from build123d import *

# Parameters (mm, degrees)
SKETCH2_R               = 32.5
CUT_EXTRUDE1_DEPTH      = 50
SKETCH3_R               = 30
CUT_EXTRUDE2_DEPTH      = 287.147252302
CHAMFER1_SIZE           = 1.5
CHAMFER2_SIZE           = 1.5
CUT_EXTRUDE3_DEPTH      = 336.306203343
CUT_EXTRUDE3_DEPTH_BACK = 336.306203343
SKETCH4_R               = 4
SKETCH7_W               = 2.1
SKETCH7_H               = 40


with BuildPart() as part:
    # Sketch1 → Revolve1 (revolve)
    with BuildSketch(Plane.XY, mode=Mode.PRIVATE) as revolve1_sk:
        Polygon((0, 0), (0, 37.5), (25, 37.5), (25, 36.5), (28, 36.5), (28, 38), (30, 38), (30, 40), (330.5, 40), (330.5, 0), align=None)
    revolve(revolve1_sk.sketch.rotate(Axis((0, 0, 0), (-1, 0, 0)), 90), axis=Axis((0, 0, 0), (-1, 0, 0)))

    # Sketch2 → Cut-Extrude1 (cut)
    with BuildSketch(Plane(origin=(330.5, 0, 0), x_dir=(0, 0, -1), z_dir=(1, 0, 0))):
        Circle(SKETCH2_R)
    extrude(amount=-CUT_EXTRUDE1_DEPTH, mode=Mode.SUBTRACT)

    # Sketch3 → Cut-Extrude2 (cut, through all)
    with BuildSketch(Plane(origin=(280.5, 0, 0), x_dir=(0, 0, -1), z_dir=(1, 0, 0))):
        Circle(SKETCH3_R)
    extrude(amount=-CUT_EXTRUDE2_DEPTH, mode=Mode.SUBTRACT)

    # Chamfer1
    chamfer1_edges = [part.edges().sort_by_distance(p)[0] for p in [
        (280.5, 0, 32.5),
    ]]
    chamfer(chamfer1_edges, length=CHAMFER1_SIZE)

    # Chamfer2
    chamfer2_edges = [part.edges().sort_by_distance(p)[0] for p in [
        (0, 0, 30),
    ]]
    chamfer(chamfer2_edges, length=CHAMFER2_SIZE)

    # Sketch4 → Cut-Extrude3 (cut, two sides: drawn at the far end of the back side and taken through both)
    with BuildSketch(Plane.XY.offset(-CUT_EXTRUDE3_DEPTH_BACK)):
        with Locations((45, 0)):
            Circle(SKETCH4_R)
    extrude(amount=CUT_EXTRUDE3_DEPTH + CUT_EXTRUDE3_DEPTH_BACK, mode=Mode.SUBTRACT)

    # Sketch7 → M5 Tapped Hole2 (revolve, cut)
    with BuildSketch(Plane.YZ.offset(323)):
        with Locations((1.05, 20)):
            Rectangle(SKETCH7_W, SKETCH7_H)
    revolve(axis=Axis((323, 0, -6.35), (0, 0, 1)), mode=Mode.SUBTRACT)


solid = part.part
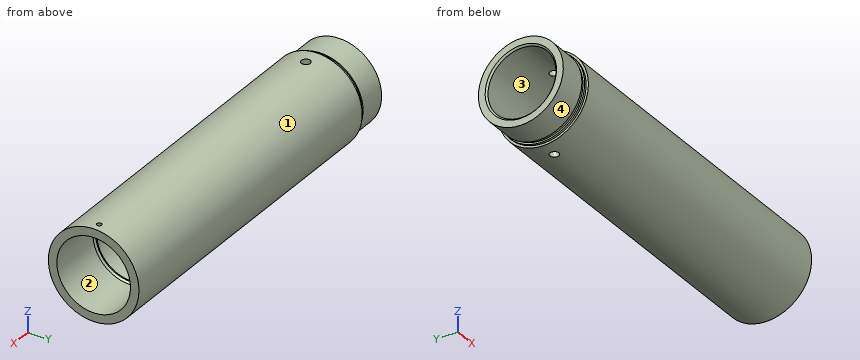
The model under review builds one solid part; all positions refer to its coordinate system, in mm. Face numbers are marked on the shaded views. A direction names the side the tool comes from. Give positions to 0.01 mm unless a question says otherwise; leave off trailing zeros. Write each loop counter-clockwise with the first axis right and the second up, starting at its lowest first coordinate (ties: lowest second). Pieces come first, ordered by that corner, then holes.
1. Add section C-C, the plane x = 261. Write out the cut boundary in (y, z).
2. Draft analysis for pull direction Y (two halves, no side actions). For the marked faces 1 and 2, state which applies: +Y half, -Y half, draft (parallel to the pull), parting line (faces both ways), or undercut.
3. Wall thickness on L1, parallel to X at y = 0, z = 36; L2, parallel to Y at x = 313, z = 0; L3, parallel to X at y = 0, z = -34.5: over which ranges is each line inside the solid? List them lowest first.
4. Add section A-A, the plane z = 0. Write out the cut boundary in (x, y).
5. Tool access review of the marked faces 3 and 4: name each direction out of +Z, -Z, +X, -X, +Y, -Y from which nothing blocks a thin tool from reaching the whole face with its end or side.
6. For P1, Ø12, axis at x = 92, y = 14.5, coming from the +Z side; P2, Ø4, axis at x = 261, y = 31, coming from the +Z side; P3, Ø8, axis at x = 104, y = 18.5, coming from the -Z side, all flat-tipped, find the tip position at first contact; note any pin that passes through.
7. Add section B-B, the plane x = 45. Write out the cut boundary in (y, z).
Worked answers:
1. outline: circle Ø80 at (0, 0); hole circle Ø60 at (0, 0)
2. face 1: parting line
2. face 2: undercut
3. L1: x = 0 to 41, 49 to 320.9, 325.1 to 330.5
3. L2: y = -40 to -32.5, 32.5 to 40
3. L3: x = 0 to 41, 49 to 330.5
4. outline: (0, -37.5) - (25, -37.5) - (25, -36.5) - (28, -36.5) - (28, -38) - (30, -38) - (30, -40) - (330.5, -40) - (330.5, -32.5) - (282, -32.5) - (280.5, -31) - (280.5, -30) - (1.5, -30) - (0, -31.5) - close; (0, 31.5) - (1.5, 30) - (280.5, 30) - (280.5, 31) - (282, 32.5) - (330.5, 32.5) - (330.5, 40) - (30, 40) - (30, 38) - (28, 38) - (28, 36.5) - (25, 36.5) - (25, 37.5) - (0, 37.5) - close
5. face 3: +X, -X
5. face 4: -X
6. P1: stops at z = 39.09
6. P2: stops at z = 27.55
6. P3: stops at z = -37.28
7. outline: (-4, -39.8) - (-4, -29.73) arc R30 cw to (-4, 29.73) - (-4, 39.8) arc R40 ccw to start; (4, -39.8) arc R40 ccw to (4, 39.8) - (4, 29.73) arc R30 cw to (4, -29.73) - close
